Input: part model. Units: mm. Frame: model coordinates. A direction names the side the tool comes from. Give positions to 0.01 mm unless a question says otherwise; leave off trailing zeros. Loops run counter-clockwise (first coordinate to the right, second up) from the corner with the lowest first, then second, coordinate; pieces in that order, holes last. Notation, with made-up numbers: M -27,84.25 L -6,84.25 A29 cw -6,113.25 Z; hole C 5,83 d2. An arc over 180 degrees is marked long. Answer as a JSON object with one key per item and string values. Group by question number.
1) Section query C-C on z = -4. Return loops of the section in (x, y).
2) Section query A-A on x = 12.75. Return loops of the section in (y, z).
3) Section query D-D on z = 0. Count the separate pieces of the cut face and the enclosed holes in it, plus the area to 3 significant figures.
4) Section query B-B on y = 13.5. Return loops of the section in (x, z).
5) First-contact query: P1, Ø1, axis at x = 7, z = -1.5, coming from the +Y side; P2, Ø5, axis at y = 17, z = 2, coming from the +X side; P3, Ø6, axis at y = 21, z = -2, coming from the +X side. Flat tips, straight axial feed; report the tip coordinate or a pass-through.
6) Draft query along Y for faces 4 (the flat face through (16.5, 37, 1.2)), 5 (the cylindrical face through (19.265, 1.014, 0.806)), 6 (the cylindrical face through (2.54, 9.56, 0.54)), 7 (the flat face through (14, 34, 0)). Return one class per face: +Y half, -Y half, draft (parallel to the pull), parting line (faces both ways), or undercut.
7) Access query for faces 1 (the flat face through (13, 0, 0)), 2 (the flat face through (10, 5, 0)), 3 (the flat face through (14, 4, 0)). Directions: +Z, -Z, +X, -X, +Y, -Y. A direction counts if a zero-diameter tool reaches every point of the face in a straight line with its end or side. Return the directions, or none.
8) Ray query, L1, parallel to Y at x = 13.25, z = -0.25; L2, parallel to Y at x = 19.75, z = 1.5; L3, parallel to X at y = 4, z = -3.75. Return the intervals inside material, ascending.
from build123d import *

# Parameters (mm, degrees)
C_BRACKET_BODY_DEPTH      = 5
WEB_HOLE_SKETCH_R         = 2.5
WEB_HOLE_DEPTH            = 10
FLANGE_HOLE_SKETCH_R      = 1.5
FLANGE_THROUGH_HOLE_DEPTH = 51


with BuildPart() as part:
    # Bracket Profile Sketch → C Bracket Body (new, symmetric)
    with BuildSketch(Plane.XY):
        with BuildLine():
            Line((0, 0), (0, 25))
            Line((0, 25), (8.238636364, 37))
            Line((8.238636364, 37), (25, 37))
            Line((25, 37), (25, 32))
            Line((25, 32), (22, 32))
            Line((22, 32), (22, 35))
            Line((22, 35), (14, 35))
            Line((14, 35), (14, 32))
            Line((14, 32), (11.923724939, 32))
            ThreePointArc((11.923724939, 32), (10.992058242, 31.769744944), (10.274912513, 31.131997167))
            Line((10.274912513, 31.131997167), (5.351187575, 23.960337118))
            ThreePointArc((5.351187575, 23.960337118), (5.08981351, 23.420950764), (5, 22.828339951))
            Line((5, 22.828339951), (5, 7))
            ThreePointArc((5, 7), (5.585786438, 5.585786438), (7, 5))
            Line((7, 5), (14, 5))
            Line((14, 5), (14, 2))
            Line((14, 2), (22, 2))
            Line((22, 2), (22, 5))
            Line((22, 5), (25, 5))
            Line((25, 5), (25, 0))
            Line((25, 0), (0, 0))
        make_face()
    extrude(amount=C_BRACKET_BODY_DEPTH, both=True)

    # Web Hole Sketch → Web Hole (cut)
    with BuildSketch(Plane(origin=(5, 0, 0), x_dir=(0, 0, -1), z_dir=(1, 0, 0))):
        with Locations((0, 12)):
            Circle(WEB_HOLE_SKETCH_R)
    extrude(amount=-WEB_HOLE_DEPTH, mode=Mode.SUBTRACT)

    # Flange Hole Sketch → Flange Through Hole (cut)
    with BuildSketch(Plane(origin=(0, 37, 0), x_dir=(1, 0, 0), z_dir=(0, 1, 0))):
        with Locations(Location((18, 0, 0), (0, 0, 270))):
            Circle(FLANGE_HOLE_SKETCH_R)
    extrude(amount=-FLANGE_THROUGH_HOLE_DEPTH, mode=Mode.SUBTRACT)


solid = part.part
Output:
{
 "1": {"outline": "M 0,0 L 25,0 L 25,5 L 22,5 L 22,2 L 14,2 L 14,5 L 7,5 A2 cw 5,7 L 5,22.83 A2 cw 5.35,23.96 L 10.27,31.13 A2 cw 11.92,32 L 14,32 L 14,35 L 22,35 L 22,32 L 25,32 L 25,37 L 8.24,37 L 0,25 Z"},
 "2": {"outline": "M 0,-5 L 5,-5 L 5,5 L 0,5 Z; M 32,-5 L 37,-5 L 37,5 L 32,5 Z"},
 "3": {"separate pieces": "4", "enclosed holes": "0", "area": "277 mm^2"},
 "4": {"outline": "M 0,-5 L 5,-5 L 5,-2 L 0,-2 Z; M 0,2 L 5,2 L 5,5 L 0,5 Z"},
 "5": {"P1": "stops at y = 35.92", "P2": "stops at x = 5", "P3": "stops at x = 5.38"},
 "6": {"face 4": "+Y half", "face 5": "draft", "face 6": "undercut", "face 7": "undercut"},
 "7": {"face 1": "+Z, -Z, +X, -X, -Y", "face 2": "+Z, -Z, +X", "face 3": "+Z, -Z"},
 "8": {"L1": "y = 0 to 5, 32 to 37", "L2": "y = 0 to 2, 35 to 37", "L3": "x = 0 to 14, 22 to 25"}
}
